CAD build for the part. Positions are in the model's coordinates, mm. A direction names the side the tool comes from. Round coordinates to 2 decimals unless told otherwise and drop trailing zeros. Loops run counter-clockwise (first coordinate to the right, second up) from the corner with the lowest first, then second, coordinate; pieces in that order, holes last.
from build123d import *

# Parameters (mm, degrees)
CHAMFER1_SIZE      = 3
M12_TAPPED_HOLE1_D = 10.2
CUT_EXTRUDE1_REACH = 95.941
SKETCH6_W          = 12
SKETCH6_H          = 6.6


with BuildPart() as part:
    # Sketch2 → Revolve1 (revolve)
    with BuildSketch(Plane.XY, mode=Mode.PRIVATE) as revolve1_sk:
        Polygon((21.5, 75), (21.5, 0), (40, 0), (40, 50), (37, 50), (37, 75), align=None)
    revolve(revolve1_sk.sketch.rotate(Axis((0, 75, 0), (0, -1, 0)), 180), axis=Axis((0, 75, 0), (0, -1, 0)))

    # Chamfer1
    chamfer1_edges = [part.edges().sort_by_distance(p)[0] for p in [
        (37, 75, 0),
    ]]
    chamfer(chamfer1_edges, length=CHAMFER1_SIZE)

    # M12 Tapped Hole1 (through all)
    with Locations(Plane(origin=(40, 0, 0), x_dir=(0, 0, -1), z_dir=(1, 0, 0))):
        with Locations((0, 20)):
            Hole(M12_TAPPED_HOLE1_D / 2)

    # Sketch6 → Cut-Extrude1 (cut, up to next)
    with BuildSketch(Plane(origin=(0, 75, 0), x_dir=(1, 0, 0), z_dir=(0, 1, 0)), mode=Mode.PRIVATE) as cut_extrude1_sk1:
        with Locations((0, -21.5)):
            Rectangle(SKETCH6_W, SKETCH6_H)
    cut_extrude1_tool1 = extrude(cut_extrude1_sk1.sketch, amount=-CUT_EXTRUDE1_REACH, mode=Mode.PRIVATE) & part.part
    add(cut_extrude1_tool1.solids().sort_by_distance((0, 75, 21.5))[0], mode=Mode.SUBTRACT)


solid = part.part
Item 1: Cut at B-B (y = 70). List the corners of the cut face in (x, z).
Verdict:
outline: circle Ø74 at (0, 0); hole (-6, 20.65) arc R21.5 ccw (long way) to (6, 20.65) - (6, 24.8) - (-6, 24.8) - close
Item 2: Flat gauge pins, fed straight in: P1, Ø4, axis at x = 10, z = 17.5, coming from the -Y side; P2, Ø5, axis at y = 49, z = -16.5, coming from the -X side; P3, Ø6, axis at y = 37.5, z = -21.5, coming from the +X side; P4, Ø2, axis at y = 30, z = 21.5, coming from the -X side. Where does each tip first touch, or does it go through?
Verdict:
P1: stops at y = 0
P2: stops at x = -37.47
P3: stops at x = 35.46
P4: stops at x = -34.35
Item 3: Cut at A-A (x = 0). List the corners of the cut face in (y, z).
Verdict:
outline: (0, -40) - (50, -40) - (50, -37) - (72, -37) - (75, -34) - (75, -21.5) - (0, -21.5) - close; (0, 24.8) - (75, 24.8) - (75, 34) - (72, 37) - (50, 37) - (50, 40) - (0, 40) - close
Item 4: 3-axis set-ups, long thin cutter, end or side, ignore diameter. For faces 1 (the cylindrical face through (30, 15, -1)), 2 (the flat face through (-11.7, 50, 35.4)), 3 (the flat face through (0, 38, 24.8)): which of +Z, -Z, +X, -X, +Y, -Y reach the whole face in a straight line?
Verdict:
face 1: +X, -X
face 2: +Y
face 3: +Y, -Y
Item 5: Mould opens along Z. For faces 4 (the flat face through (-6, 38, 23)), 5 (the flat face through (-22, 75, 0)), 6 (the cylindrical face through (-17.073, 61.154, 32.825)) say: released by +Z, released by -Z, zero draft, split by the parting line, or undercut.
Verdict:
face 4: undercut
face 5: zero draft
face 6: split by the parting line
Item 6: Wall check: L1, parallel to Y at x = 30, z = 0; L2, parallel to Z at x = 0, y = 28; L3, parallel to X at y = 66, z = -0.5. Give the ranges that are in metal, low to high.
Verdict:
L1: y = 0 to 14.9, 25.1 to 75
L2: z = -40 to -21.5, 24.8 to 40
L3: x = -37 to -21.49, 21.49 to 37
Item 7: Cut at C-C (y = 20). List the corners of the cut face in (x, z), plus the area to 3 significant figures.
Verdict:
outline: (-39.67, -5.1) arc R40 ccw to (39.67, -5.1) - (20.89, -5.1) arc R21.5 cw to (-20.89, -5.1) - close; (-39.67, 5.1) - (-20.89, 5.1) arc R21.5 cw to (-6, 20.65) - (-6, 24.8) - (6, 24.8) - (6, 20.65) arc R21.5 cw to (20.89, 5.1) - (39.67, 5.1) arc R40 ccw to start
area: 3,150 mm2
